Can you work these out from the model? Positions are in its coordinate system, mm. Round coordinates to 2 decimals unless told otherwise and drop trailing zeros. Loops run counter-clockwise (first coordinate to the right, second up) from the corner with the lowest first, then second, coordinate; pieces in that order, holes last. Notation, with made-up numbers: M 33.5,50.5 L 66.5,50.5 A27 cw 66.5,73.5 Z; hole C 20,9 d3. An arc over 180 degrees is marked long. Return JSON: item names as keys, results as strings.
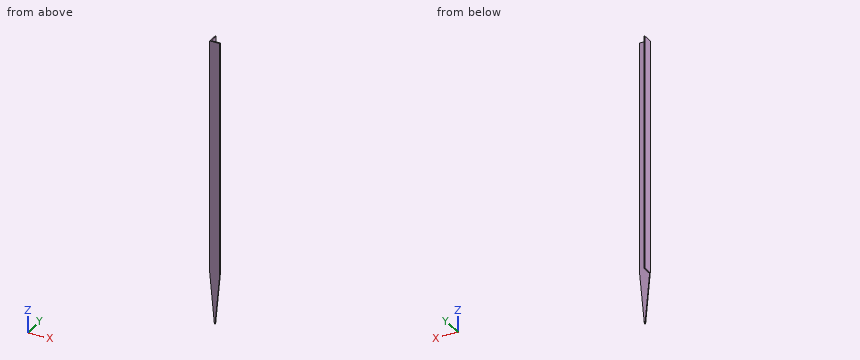
```python
from build123d import *

# Parameters (mm, degrees)
EXTRUDE1_DEPTH = 1295.4
EXTRUDE2_DEPTH = 1297.627083248
SKETCH5_W      = 54.662840746
SKETCH5_H      = 40
EXTRUDE3_DEPTH = 1297.759359805


with BuildPart() as part:
    # Sketch1 → Extrude1 (new body)
    with BuildSketch(Plane.XY):
        Polygon((-11.005397301, 1.140254873), (-11.005397301, -43.859745127), (33.994602699, -43.859745127), (33.994602699, -38.859745127), (-6.005397301, -38.859745127), (-6.005397301, 1.140254873), align=None)
    extrude(amount=EXTRUDE1_DEPTH)

    # Sketch2 → Extrude2 (cut, through all)
    with BuildSketch(Plane.XZ.offset(43.859745127)):
        Polygon((-11.005397301, 0), (9.904602699, 0), (-11.005397301, 228.6), align=None)
        Polygon((33.994602699, 228.6), (13.084602699, 0), (33.994602699, 0), align=None)
    extrude(amount=-EXTRUDE2_DEPTH, mode=Mode.SUBTRACT)

    # Sketch5 → Extrude3 (cut, through all)
    with BuildSketch(Plane(origin=(-6.005397301, 0, 0), x_dir=(0, 0, -1), z_dir=(1, 0, 0))):
        with Locations((-201.268579627, -18.859745127)):
            Rectangle(SKETCH5_W, SKETCH5_H)
    extrude(amount=-EXTRUDE3_DEPTH, mode=Mode.SUBTRACT)


solid = part.part
```
Q1. Suppose I cut it at C-C, the plane x = 21. Please give me the cut outline in (y, z), plus the area to 3 significant figures.
Results:
{"outline": "M -43.86,86.54 L -38.86,86.54 L -38.86,1295.4 L -43.86,1295.4 Z", "area": "6,040 mm2"}
Q2. If I drill on line 1 along X through (y, z) = (-7.5, 564); line 2 along Y through (x, z) = (25.5, 786); line 3 along Z through (x, y) = (-8, -36.5), over which ranges is the centre line in solid material (lowest first)?
Results:
{"line 1": "x = -11.01 to -6.01", "line 2": "y = -43.86 to -38.86", "line 3": "z = 228.6 to 1295.4"}
Q3. I'm going to push flat-ended pins straight in: pin 1 Ø6 at (y, z) = (-34, 299.5) entering from +X; pin 2 Ø5 at (x, z) = (21, 185) entering from +Y; pin 3 Ø1.5 at (x, y) = (-8, -15.5) entering from -Z. Where does each tip first touch, or does it pass through?
Results:
{"pin 1": "stops at x = -6.01", "pin 2": "stops at y = -38.86", "pin 3": "stops at z = 228.6"}
Q4. Suppose I cut it at B-B, the plane z = 1077.5. Please give me the cut outline in (x, y), plus the area to 3 significant figures.
Results:
{"outline": "M -11.01,-43.86 L 33.99,-43.86 L 33.99,-38.86 L -6.01,-38.86 L -6.01,1.14 L -11.01,1.14 Z", "area": "425 mm2"}
Q5. Suppose I cut it at A-A, the plane y = -21.5. Please give me the cut outline in (x, z).
Results:
{"outline": "M -11.01,228.6 L -6.01,228.6 L -6.01,1295.4 L -11.01,1295.4 Z"}
